```python
from build123d import *

# Parameters (mm, degrees)
BOSS_EXTRUDE1_DEPTH = 6
CHAMFER1_SIZE       = 4
CHAMFER1_SIZE2      = 4.024049749


with BuildPart() as part:
    # Sketch1 → Boss-Extrude1 (new body)
    with BuildSketch(Plane.XY):
        Polygon((0, 0), (0, 60), (68.372865684, 50.718230869), (64, 17), (10, 0), align=None)
    extrude(amount=BOSS_EXTRUDE1_DEPTH)

    # Chamfer1
    chamfer1_edges = [part.edges().sort_by_distance(p)[0] for p in [
        (68.372865684, 50.718230869, 3),
    ]]
    chamfer1_side = [part.faces().sort_by_distance(p)[0] for p in [
        (66.186432842, 33.859115434, 3),
    ]]
    chamfer(chamfer1_edges, length=CHAMFER1_SIZE, length2=CHAMFER1_SIZE2, reference=chamfer1_side[0])


solid = part.part
```
For this review, take the finished solid that the model builds, in its own axes (mm). Round coordinates to 2 decimals unless told otherwise and drop trailing zeros. Write each loop counter-clockwise with the first axis right and the second up, starting at its lowest first coordinate (ties: lowest second). Pieces come first, ordered by that corner, then holes. Notation, with made-up numbers: (-24, 20) - (4, 20) arc R14 cw to (4, 39) - close; hole circle Ø8 at (1.25, 13). An arc over 180 degrees is marked (long way). Write each question's results on one line, items separated by ' | '.
Item 1: To check wall thickness, follow line 1 along X through (y, z) = (21, 4.5); line 2 along Y through (x, z) = (6.5, 0.35); line 3 along Y through (x, z) = (37.5, 0.65). State the ranges of each line that lie inside material, in increasing order. Write a range as from..to.
Calculated:
line 1: x = 0..64.52 | line 2: y = 0..59.12 | line 3: y = 8.66..54.91
Item 2: Take a section at A-A on z = 2.3. State the section outline as (x, y) points, then the cut area to 3 significant figures.
Calculated:
outline: (0, 0) - (10, 0) - (64, 17) - (67.86, 46.75) - (64.39, 51.26) - (0, 60) - close | area: 3,170 mm^2
Item 3: Take a section at C-C on x = 41. State the section outline as (y, z) points.
Calculated:
outline: (9.76, 0) - (54.43, 0) - (54.43, 6) - (9.76, 6) - close
Item 4: For pin 1 (1 mm diameter, centred on y = 50.5, z = 1.5, fed in from +X); pin 2 (2 mm diameter, centred on y = 36, z = 5, fed in from +X); pin 3 (1 mm diameter, centred on y = 37, z = 4, fed in from -X), all flat-tipped, find the tip position at first contact; note any pin that passes through.
Calculated:
pin 1: stops at x = 65.36 | pin 2: stops at x = 66.59 | pin 3: stops at x = 0
Item 5: Take a section at B-B on y = 54.5. State the section outline as (x, z) points, then the cut area to 3 significant figures.
Calculated:
outline: (0, 0) - (40.51, 0) - (40.51, 6) - (0, 6) - close | area: 243 mm^2
